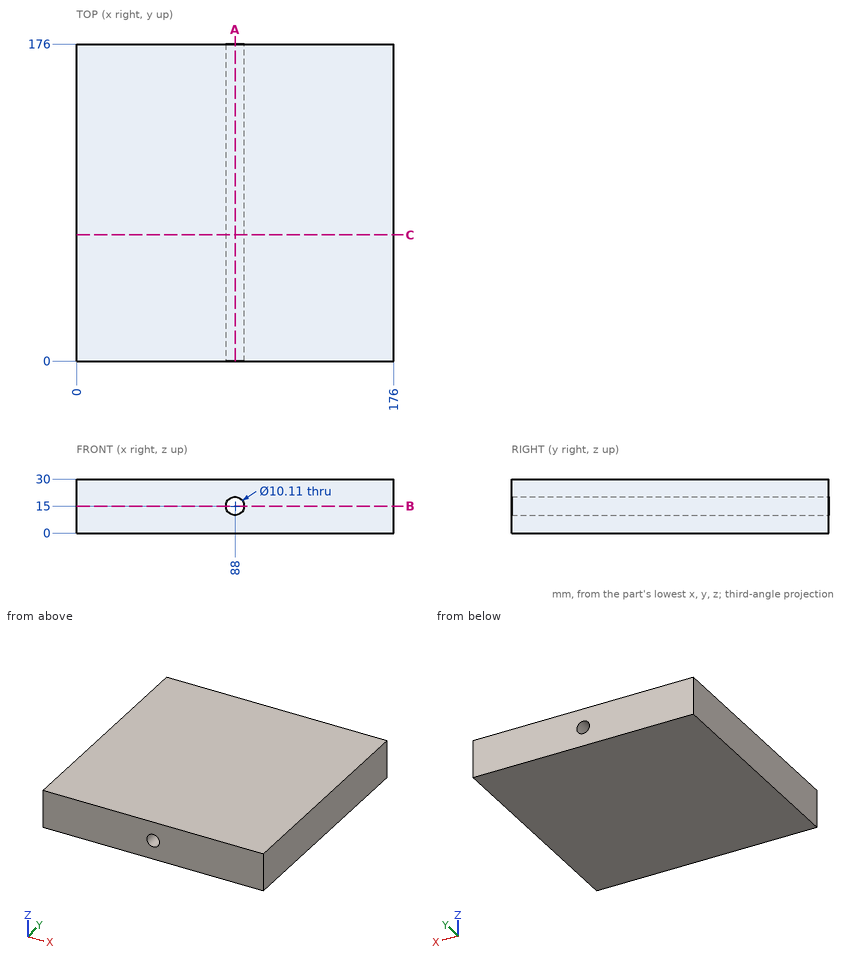
Design review of the part shown in the three views and the two pictorial views. Dimensions are in mm from the part's minimum x, y and z. Give positions to 0.01 mm unless a question says otherwise; leave off trailing zeros. Write each loop counter-clockwise with the first axis right and the second up, starting at its lowest first coordinate (ties: lowest second). Pieces come first, ordered by that corner, then holes.
Item 1: Take a section at B-B (z = 15). Give the boundary of the cut face in (x, y) (3 decimals).
Item 2: Take a section at A-A (x = 88). Give the boundary of the cut face in (y, z) (3 decimals).
Item 3: Wall thickness on probe 1 along X at (y, z) = (90.5, 15.5); probe 2 along Z at (x, y) = (88, 36) (3 decimals); probe 3 along X at (y, z) = (159, 10.5): over which ranges is each line inside the solid? List them lowest first.
Item 4: Take a section at C-C (y = 70). Give the boundary of the cut face in (x, z) (3 decimals), and give its area (3 significant figures).
Established:
1. outline: (0, 0) - (82.945, 0) - (82.945, 176) - (0, 176) - close; (93.055, 0) - (176, 0) - (176, 176) - (93.055, 176) - close
2. outline: (0, 0) - (176, 0) - (176, 9.945) - (0, 9.945) - close; (0, 20.055) - (176, 20.055) - (176, 30) - (0, 30) - close
3. probe 1: x = 0 to 82.97, 93.03 to 176
3. probe 2: z = 0 to 9.945, 20.055 to 30
3. probe 3: x = 0 to 85.7, 90.3 to 176
4. outline: (0, 0) - (176, 0) - (176, 30) - (0, 30) - close; hole circle Ø10.11 at (88, 15)
4. area: 5,200 mm2
